Read the model definition and answer for the solid it produces. Units are mm, in the model's axes. A direction names the side the tool comes from. Give positions to 0.01 mm unless a question says otherwise; leave off trailing zeros. Write each loop counter-clockwise with the first axis right and the second up, starting at its lowest first coordinate (ties: lowest second). Pieces come first, ordered by that corner, then holes. Notation, with made-up numbers: (23, 70) -> (47, 70) arc R11 cw to (47, 90) -> close; hole circle Ø6 at (88, 66). An arc over 180 degrees is marked (long way). Answer as CSV lines item,"result". Start each with the question number.
1. The part is cut by section A-A, the plane y = 7.75. Determine the outline of the cut face in (x, z), and give its area (3 significant figures).
2. For a pull along Z with two mould halves and no side action, classify faces 4 (the flat face through (0, 9.5, 3)), 5 (the cylindrical face through (-4.88, 2.96, -1.08)), 6 (the flat face through (2.155, 7.035, 1.267)) as pulls with the +Z half, pulls with the -Z half, needs draft (parallel to the pull), parting line crosses it, or undercut.
3. The part is cut by section B-B, the plane x = 0. Determine the outline of the cut face in (y, z).
4. Find the intervals of material crossed by line 1 (Y direction, x = 5.75, z = -3); line 2 (X direction, y = 8.25, z = 2); line 3 (X direction, y = 5, z = 1), in increasing order.
5. The part is cut by section C-C, the plane y = 9.25. Determine the outline of the cut face in (x, z).
6. Given pin 1 (2 mm diameter, centred on x = -3.5, y = 4.5, fed in from -Z); pin 2 (1 mm diameter, centred on x = -3.5, y = 4, fed in from -Z), each flat-ended and moving along its own axis, determine where each tip first touches the part or whether it passes through.
7. A tool of negligible diameter and unlimited length cuts with its end or side. For faces 1 (the cylindrical face through (-6.834, 7.571, -1.517)), 2 (the flat face through (-5, 6, 2)), 3 (the flat face through (0, 7, 2.5)), from which of +Z, -Z, +X, -X, +Y, -Y can it reach the whole face along a straight path? Write none if from no direction.
from build123d import *
from OCP.BRepFilletAPI import BRepFilletAPI_MakeChamfer

# Parameters (mm, degrees)
SKETCH1_R           = 5
BOSS_EXTRUDE1_DEPTH = 6
SKETCH3_R           = 7
BOSS_EXTRUDE2_DEPTH = 3.5
CUT_EXTRUDE1_DEPTH  = 5
CHAMFER1_SIZE       = 0.5
CHAMFER1_SIZE2      = 0.181985117


with BuildPart() as part:
    # Sketch1 → Boss-Extrude1 (new body)
    with BuildSketch(Plane(origin=(0, 0, 0), x_dir=(1, 0, 0), z_dir=(0, 1, 0))):
        with Locations(Location((0, 0, 0), (0, 0, 270))):
            Circle(SKETCH1_R)
    extrude(amount=BOSS_EXTRUDE1_DEPTH)

    # Sketch3 → Boss-Extrude2 (add)
    with BuildSketch(Plane(origin=(0, 6, 0), x_dir=(1, 0, 0), z_dir=(0, 1, 0))):
        with Locations(Location((0, 0, 0), (0, 0, 270))):
            Circle(SKETCH3_R)
    extrude(amount=BOSS_EXTRUDE2_DEPTH)

    # Sketch4 → Cut-Extrude1 (cut)
    with BuildSketch(Plane(origin=(0, 9.5, 0), x_dir=(1, 0, 0), z_dir=(0, 1, 0))):
        Polygon((-2.886751346, 0), (-1.443375673, -2.5), (1.443375673, -2.5), (2.886751346, 0), (1.443375673, 2.5), (-1.443375673, 2.5), align=None)
    extrude(amount=-CUT_EXTRUDE1_DEPTH, mode=Mode.SUBTRACT)

    # Chamfer1: one chamfer whose edges measure the first distance from different faces: ONE call of the kernel's chamfer builder (chamfer() names one face for all edges)
    chamfer1_edges_1 = [part.edges().sort_by_distance(p)[0] for p in [
        (0, 6, -7),
    ]]
    chamfer1_side_1 = [part.faces().sort_by_distance(p)[0] for p in [
        (0, 6, -6.802010101),
    ]]
    chamfer1_edges_2 = [part.edges().sort_by_distance(p)[0] for p in [
        (0, 9.5, -7),
    ]]
    chamfer1_side_2 = [part.faces().sort_by_distance(p)[0] for p in [
        (0, 7.75, -7),
    ]]
    chamfer1 = BRepFilletAPI_MakeChamfer(part.part.solid().wrapped)
    for e in chamfer1_edges_1:
        chamfer1.Add(CHAMFER1_SIZE, CHAMFER1_SIZE2, e.wrapped, chamfer1_side_1[0].wrapped)  # the first distance lies on this face
    for e in chamfer1_edges_2:
        chamfer1.Add(CHAMFER1_SIZE, CHAMFER1_SIZE2, e.wrapped, chamfer1_side_2[0].wrapped)  # the first distance lies on this face
    add(Compound.cast(chamfer1.Shape()), mode=Mode.REPLACE)


solid = part.part
Results found:
1,outline,"circle Ø14 at (0, 0); hole (-2.89, 0) -> (-1.44, -2.5) -> (1.44, -2.5) -> (2.89, 0) -> (1.44, 2.5) -> (-1.44, 2.5) -> close"
1,area,"132 mm²"
2,face 4,"needs draft"
2,face 5,"parting line crosses it"
2,face 6,"undercut"
3,outline,"(0, -5) -> (6, -5) -> (6, -6.5) -> (6.18, -7) -> (9, -7) -> (9.5, -6.82) -> (9.5, -2.5) -> (4.5, -2.5) -> (4.5, 2.5) -> (9.5, 2.5) -> (9.5, 6.82) -> (9, 7) -> (6.18, 7) -> (6, 6.5) -> (6, 5) -> (0, 5) -> close"
4,line 1,"y = 6 to 9.5"
4,line 2,"x = -6.71 to -1.73, 1.73 to 6.71"
4,line 3,"x = -4.9 to -2.31, 2.31 to 4.9"
5,outline,"circle Ø13.82 at (0, 0); hole (-2.89, 0) -> (-1.44, -2.5) -> (1.44, -2.5) -> (2.89, 0) -> (1.44, 2.5) -> (-1.44, 2.5) -> close"
6,pin 1,"stops at z = -4.33"
6,pin 2,"stops at z = -4"
7,face 1,"+Y, -Y"
7,face 2,"-Y"
7,face 3,"+Y"
